from build123d import *

# Parameters (mm, degrees)
EXTRUDE_THIN1_DEPTH = 548.8


with BuildPart() as part:
    # Sketch1 → Extrude-Thin1 (new, symmetric)
    with BuildSketch(Plane.XY):
        with BuildLine():
            Line((-15, 11), (-15, -11))
            ThreePointArc((-15, -11), (-13.828427125, -13.828427125), (-11, -15))
            Line((-11, -15), (11, -15))
            ThreePointArc((11, -15), (13.828427125, -13.828427125), (15, -11))
            Line((15, -11), (15, 11))
            ThreePointArc((15, 11), (13.828427125, 13.828427125), (11, 15))
            Line((11, 15), (-11, 15))
            ThreePointArc((-11, 15), (-13.828427125, 13.828427125), (-15, 11))
        make_face()
        with BuildLine():
            Line((-13, 11), (-13, -11))
            ThreePointArc((-13, -11), (-12.414213562, -12.414213562), (-11, -13))
            Line((-11, -13), (11, -13))
            ThreePointArc((11, -13), (12.414213562, -12.414213562), (13, -11))
            Line((13, -11), (13, 11))
            ThreePointArc((13, 11), (12.414213562, 12.414213562), (11, 13))
            Line((11, 13), (-11, 13))
            ThreePointArc((-11, 13), (-12.414213562, 12.414213562), (-13, 11))
        make_face(mode=Mode.SUBTRACT)
    extrude(amount=EXTRUDE_THIN1_DEPTH, both=True)


solid = part.part
Read the model definition and answer for the solid it produces. Units are mm, in the model's axes. A direction names the side the tool comes from. Give positions to 0.01 mm unless a question says otherwise; leave off trailing zeros. Write each loop counter-clockwise with the first axis right and the second up, starting at its lowest first coordinate (ties: lowest second). Pieces come first, ordered by that corner, then holes. Notation, with made-up numbers: M 82,-38 L 120,-38 A26 ccw 120,-10 Z; hole C -39.75,73.5 d4. An arc over 180 degrees is marked long. One line per item, written item: value. Start each with the question number.
(1) A tool of negligible diameter and unlimited length cuts with its end or side. For faces 4 (the flat face through (0, -13, 8)), 5 (the flat face through (15, 0, 8)), from which of +Z, -Z, +X, -X, +Y, -Y can it reach the whole face along a straight path? Write none if from no direction.
(2) Find section C-C (z = -310.5). Determine the outline of the cut face in (x, y).
(3) Flat-ended cylindrical pins translate along their axes: pin 1 Ø12 at (x, y) = (-0.5, -10) entering from -Z; pin 2 Ø8 at (x, y) = (4.5, 7) entering from +Z. Find the tip coordinate at first contact, or state that the pin passes through.
(4) Find section A-A (y = -2.75). Determine the outline of the cut face in (x, z), plus the area to 3 significant figures.
(5) Determine the mould class of faces 1 (the flat face through (13, 0, 8)), 2 (the flat face through (0, -15, 8)), 3 (the flat face through (-15, 0, 8)) for opening direction Y: pulls with the +Y half, pulls with the -Y half, needs draft (parallel to the pull), parting line crosses it, or undercut.
(6) Find the intervals of material crossed by line 1 (X direction, y = -4, z = 412); line 2 (X direction, y = -11.75, z = 186.5); line 3 (Y direction, x = -11.5, z = -352.5), in increasing order.
Results below:
1. face 4: +Z, -Z
1. face 5: +Z, -Z, +X, +Y, -Y
2. outline: M -15,-11 A4 ccw -11,-15 L 11,-15 A4 ccw 15,-11 L 15,11 A4 ccw 11,15 L -11,15 A4 ccw -15,11 Z; hole M -13,-11 A2 ccw -11,-13 L 11,-13 A2 ccw 13,-11 L 13,11 A2 ccw 11,13 L -11,13 A2 ccw -13,11 Z
3. pin 1: stops at z = -548.8
3. pin 2: passes through
4. outline: M -15,-548.8 L -13,-548.8 L -13,548.8 L -15,548.8 Z; M 13,-548.8 L 15,-548.8 L 15,548.8 L 13,548.8 Z
4. area: 4,390 mm^2
5. face 1: undercut
5. face 2: pulls with the -Y half
5. face 3: needs draft
6. line 1: x = -15 to -13, 13 to 15
6. line 2: x = -14.93 to -12.85, 12.85 to 14.93
6. line 3: y = -14.97 to -12.94, 12.94 to 14.97
